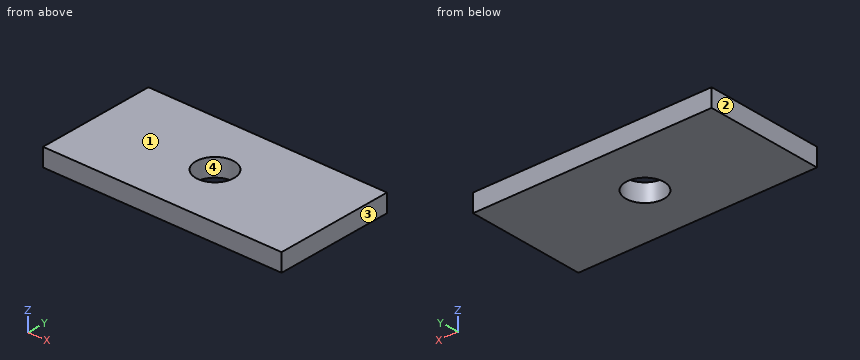
from build123d import *

# Parameters (mm, degrees)
SKETCH_1_W          = 40
SKETCH_1_H          = 20
EXTRUDE_1_DEPTH     = 1.5
SKETCH_2_R          = 3.2
CUT_EXTRUDE_1_DEPTH = 11.5


with BuildPart() as part:
    # 草图1 → 凸台-拉伸1 (new, symmetric)
    with BuildSketch(Plane.XY):
        Rectangle(SKETCH_1_W, SKETCH_1_H)
    extrude(amount=EXTRUDE_1_DEPTH, both=True)

    # 草图2 → 切除-拉伸1 (cut, symmetric)
    with BuildSketch(Plane.XY):
        Circle(SKETCH_2_R)
    extrude(amount=CUT_EXTRUDE_1_DEPTH, both=True, mode=Mode.SUBTRACT)


solid = part.part
Build history of the part. All positions in model axes, mm. Face numbers are marked on the shaded views. Give positions to 0.01 mm unless a question says otherwise; leave off trailing zeros. Order: outer loops, then holes, each group sorted by start corner. A loop starts at its lowest first (then second) coordinate and runs counter-clockwise, first axis right, second up. Notation, with made-up numbers: M -21,24 L 19,24 A9 cw 19,33 Z; hole C 54.25,47.5 d4. An arc over 180 degrees is marked long. Use one line per item in the form item = value.
1) Saw through at C-C (z = 0.8). Give the cut face in (x, y).
Calculated:
outline = M -20,-10 L 20,-10 L 20,10 L -20,10 Z; hole C 0,0 d6.4
2) Saw through at B-B (y = 0). Give the cut face in (x, z).
Calculated:
outline = M -20,-1.5 L -3.2,-1.5 L -3.2,1.5 L -20,1.5 Z; M 3.2,-1.5 L 20,-1.5 L 20,1.5 L 3.2,1.5 Z
3) Saw through at A-A (x = 0). Give the cut face in (y, z), plus the area to 3 significant figures.
Calculated:
outline = M -10,-1.5 L -3.2,-1.5 L -3.2,1.5 L -10,1.5 Z; M 3.2,-1.5 L 10,-1.5 L 10,1.5 L 3.2,1.5 Z
area = 40.8 mm2
4) Probe probe 1 along Y at (x, z) = (0, -0.2); probe 2 along Y at (x, z) = (1.5, 0.9); probe 3 along X at (y, z) = (2.5, 0.8). List the from-to ranges inside material, lowest first.
Calculated:
probe_1 = -10 to -3.2, 3.2 to 10
probe_2 = -10 to -2.83, 2.83 to 10
probe_3 = -20 to -2, 2 to 20
5) Two-plate mould, pull along X, no slides. Class the marked faces 1, 2, 3 and 4: released by +X, released by -X, zero draft, split by the parting line, or undercut.
Calculated:
face_1 = zero draft
face_2 = released by -X
face_3 = released by +X
face_4 = undercut
